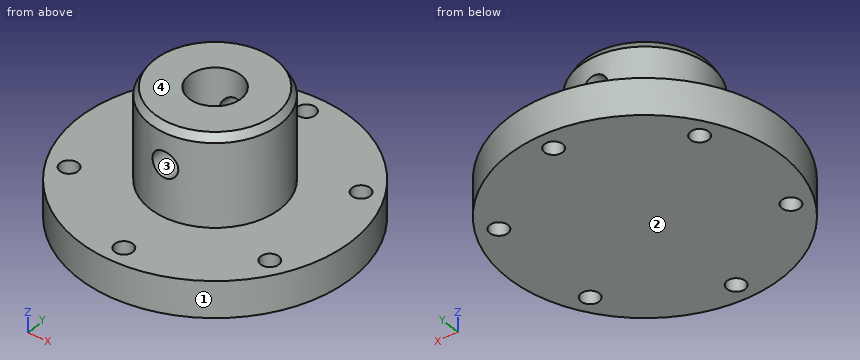
```python
from build123d import *

# Parameters (mm, degrees)
SKETCH1_R               = 52.5
SKETCH1_R_2             = 3.5
BOSS_EXTRUDE1_DEPTH     = 14
SKETCH2_R               = 25
SKETCH2_R_2             = 10
BOSS_EXTRUDE2_DEPTH     = 35
CUT_EXTRUDE1_DEPTH      = 89.95785519
CUT_EXTRUDE1_DEPTH_BACK = 89.95785519
SKETCH3_R               = 5
CHAMFER1_SIZE           = 3
CHAMFER1_SIZE2          = 1.732050808


with BuildPart() as part:
    # Sketch1 → Boss-Extrude1 (new body)
    with BuildSketch(Plane.XY):
        Circle(SKETCH1_R)
        with Locations((0, 45)):
            Circle(SKETCH1_R_2, mode=Mode.SUBTRACT)
        with Locations((38.97114317, 22.5)):
            Circle(SKETCH1_R_2, mode=Mode.SUBTRACT)
        with Locations((38.97114317, -22.5)):
            Circle(SKETCH1_R_2, mode=Mode.SUBTRACT)
        with Locations((0, -45)):
            Circle(SKETCH1_R_2, mode=Mode.SUBTRACT)
        with Locations((-38.97114317, -22.5)):
            Circle(SKETCH1_R_2, mode=Mode.SUBTRACT)
        with Locations((-38.97114317, 22.5)):
            Circle(SKETCH1_R_2, mode=Mode.SUBTRACT)
    extrude(amount=BOSS_EXTRUDE1_DEPTH)

    # Sketch2 → Boss-Extrude2 (add)
    with BuildSketch(Plane.XY.offset(14)):
        Circle(SKETCH2_R)
        Circle(SKETCH2_R_2, mode=Mode.SUBTRACT)
    extrude(amount=BOSS_EXTRUDE2_DEPTH)

    # Sketch3 → Cut-Extrude1 (cut, two sides: drawn at the far end of the back side and taken through both)
    with BuildSketch(Plane(origin=(0, 0, 0), x_dir=(1, 0, 0), z_dir=(0, 1, 0)).offset(-CUT_EXTRUDE1_DEPTH_BACK)):
        with Locations(Location((0, -34, 0), (0, 0, 270))):
            Circle(SKETCH3_R)
    extrude(amount=CUT_EXTRUDE1_DEPTH + CUT_EXTRUDE1_DEPTH_BACK, mode=Mode.SUBTRACT)

    # Chamfer1
    chamfer1_edges = [part.edges().sort_by_distance(p)[0] for p in [
        (-25, 0, 49),
    ]]
    chamfer1_side = [part.faces().sort_by_distance(p)[0] for p in [
        (-25, 0, 31.5),
    ]]
    chamfer(chamfer1_edges, length=CHAMFER1_SIZE, length2=CHAMFER1_SIZE2, reference=chamfer1_side[0])


solid = part.part
```
Geometry: final body of the model. Coordinates: model frame, mm. Face numbers are marked on the shaded views. Round coordinates to 2 decimals unless told otherwise and drop trailing zeros. Write each loop counter-clockwise with the first axis right and the second up, starting at its lowest first coordinate (ties: lowest second). Pieces come first, ordered by that corner, then holes. Notation, with made-up numbers: (45, 27) -> (100, 27) arc R24 cw to (100, 50) -> close; hole circle Ø1 at (36, 67). An arc over 180 degrees is marked (long way). Return JSON: item names as keys, results as strings.
Q1. Mould query, pull axis Z, two halves, no side actions, for the marked faces 1, 2, 3 and 4. Classes: +Z half, -Z half, draft (parallel to the pull), parting line (faces both ways), or undercut.
From the geometry:
{"face 1": "draft", "face 2": "-Z half", "face 3": "undercut", "face 4": "+Z half"}
Q2. Section C-C on z = 41.5. Return the cut outline in (x, y), and give its area (3 significant figures).
From the geometry:
{"outline": "circle Ø50 at (0, 0); hole circle Ø20 at (0, 0)", "area": "1,650 mm2"}
Q3. First-contact query: pin 1 Ø8 at (y, z) = (-42, 6) entering from -X (3 decimals); pin 2 Ø2 at (y, z) = (-16, 23) entering from +X; pin 3 Ø16 at (x, z) = (0, 34) entering from -Y; pin 4 Ø9 at (x, z) = (0, 34) entering from +Y. Flat tips, straight axial feed; report the tip coordinate or a pass-through.
From the geometry:
{"pin 1": "x = -36.225", "pin 2": "x = 20", "pin 3": "y = -25", "pin 4": "through"}
Q4. Section B-B on y = -43. Return the cut outline in (x, z), and give its area (3 significant figures).
From the geometry:
{"outline": "(-30.12, 0) -> (-2.87, 0) -> (-2.87, 14) -> (-30.12, 14) -> close; (2.87, 0) -> (30.12, 0) -> (30.12, 14) -> (2.87, 14) -> close", "area": "763 mm2"}
Q5. Section D-D on z = 33. Return the cut outline in (x, y), and give its area (3 significant figures).
From the geometry:
{"outline": "(-4.9, -24.52) -> (-4.9, -8.72) arc R10 cw to (-4.9, 8.72) -> (-4.9, 24.52) arc R25 ccw to start; (4.9, -24.52) arc R25 ccw to (4.9, 24.52) -> (4.9, 8.72) arc R10 cw to (4.9, -8.72) -> close", "area": "1,350 mm2"}
Q6. Ray query, line 1 (Y direction, x = 0, z = 11); line 2 (X direction, y = -22, z = 9); line 3 (Z direction, x = 0, y = -18). Return the intervals inside material, ascending.
From the geometry:
{"line 1": "-52.5 to -48.5, -41.5 to 41.5, 48.5 to 52.5", "line 2": "-47.67 to -42.44, -35.51 to 35.51, 42.44 to 47.67", "line 3": "0 to 29, 39 to 49"}
Q7. Section A-A on x = 0. Give the number of separate pieces and of enclosed holes in the cut face, and give its area (3 significant figures).
From the geometry:
{"separate pieces": "5", "enclosed holes": "0", "area": "2,020 mm2"}
